Input: part model. Units: mm. Frame: model coordinates. A direction names the side the tool comes from. Give positions to 0.01 mm unless a question says otherwise; leave off trailing zeros. Loops run counter-clockwise (first coordinate to the right, second up) from the corner with the lowest first, then second, coordinate; pieces in that order, holes last. Notation, with made-up numbers: (-25.5, -17.75) - (-16.5, -17.75) arc R25 cw to (-16.5, -3.75) - close; hole circle Ø1 at (28.25, 75). An arc over 180 degrees is marked (long way). Answer as a JSON object with one key per item and string values. Group by question number.
(1) Access query for faces 5 (the flat face through (182, 0, -21)), 6 (the flat face through (184, -40, -5)). Directions: +Z, -Z, +X, -X, +Y, -Y. A direction counts if a zero-diameter tool reaches every point of the face in a straight line with its end or side. Return the directions, or none.
(2) Material intervals for L1, parallel to Z at x = 94.5, y = -63.5; L2, parallel to Y at x = 232, z = -37.5; L3, parallel to Y at x = 209, z = -15, sorted ascending.
(3) Pin query (flat end, axial travel): P1, Ø2, axis at x = 95.5, y = -23.5, coming from the -Z side. Return the tip coordinate at first contact, or that it passes through.
(4) Section query D-D (y = -13.5). Return loops of the section in (x, z), plus the area to 3 significant figures.
(5) Section query B-B (x = 260.5). Return loops of the section in (y, z), plus the area to 3 significant figures.
(6) Section query A-A (z = -27.5). Return loops of the section in (x, y), plus the area to 3 significant figures.
(7) Section query C-C (z = -14.5). Return loops of the section in (x, y), plus the area to 3 significant figures.
(8) Mould query, pull axis Y, two halves, no side actions, for faces 1 (the cylindrical face through (183.28, -11.711, -7.124)), 2 (the flat face through (300, -40, -4)), 3 (the flat face through (189.72, -72.16, -25.61)), 4 (the flat face through (190, -80, -22)). Classes: +Y half, -Y half, draft (parallel to the pull), parting line (faces both ways), or undercut.
```python
from build123d import *

# Parameters (mm, degrees)
GB_T707_1988_8_XXXXXXXXXXXXXXX528V9_1_DEPTH = 300
CUT_EXTRUDE_2_REACH                         = 315.447
SKETCH_4_R                                  = 895


with BuildPart() as part:
    # Sketch11 → 热轧普通槽钢(gb t707-1988) 8-XXXXXXXXXXXXXXX528V9(1) (new body)
    with BuildSketch(Plane(origin=(0, 0, 0), x_dir=(0, 0, -1), z_dir=(-1, 0, 0))):
        with BuildLine():
            Line((43, 80), (0, 80))
            Line((0, 80), (0, 0))
            Line((0, 0), (43, 0))
            Line((43, 0), (43, 2.480049752))
            ThreePointArc((43, 2.480049752), (41.965810134, 5.164071035), (39.398014876, 6.460198512))
            Line((39.398014876, 6.460198512), (12.203970248, 9.179602975))
            ThreePointArc((12.203970248, 9.179602975), (7.068379732, 11.771857931), (5, 17.139900497))
            Line((5, 17.139900497), (5, 62.860099503))
            ThreePointArc((5, 62.860099503), (7.068379732, 68.228142069), (12.203970248, 70.820397025))
            Line((12.203970248, 70.820397025), (39.398014876, 73.539801488))
            ThreePointArc((39.398014876, 73.539801488), (41.965810134, 74.835928965), (43, 77.519950248))
            Line((43, 77.519950248), (43, 80))
        make_face()
    extrude(amount=-GB_T707_1988_8_XXXXXXXXXXXXXXX528V9_1_DEPTH)

    # 草图4 → 切除-拉伸2 (cut, up to next)
    with BuildSketch(Plane.XY, mode=Mode.PRIVATE) as cut_extrude_2_sk1:
        with Locations((-799.887205022, -220.600173536)):
            Circle(SKETCH_4_R)
    cut_extrude_2_tool1 = extrude(cut_extrude_2_sk1.sketch, amount=-CUT_EXTRUDE_2_REACH, mode=Mode.PRIVATE) & part.part
    add(cut_extrude_2_tool1.solids().sort_by_distance((-799.887205, -220.600174, 0))[0], mode=Mode.SUBTRACT)


solid = part.part
```
Recorded:
{
 "1": {"face 5": "+Z, -Z, +X, -X, +Y", "face 6": "-Z, +X, -X"},
 "2": {"L1": "z = -5.03 to 0", "L2": "y = -80 to -73.35, -6.65 to 0", "L3": "y = -80 to -71.1, -8.9 to 0"},
 "3": {"P1": "stops at z = -5"},
 "4": {"outline": "(70.82, -5.88) - (300, -5.88) - (300, 0) - (70.82, 0) - close", "area": "1,350 mm^2"},
 "5": {"outline": "(-80, -43) - (-77.52, -43) arc R4 ccw to (-73.54, -39.4) - (-70.82, -12.2) arc R8 cw to (-62.86, -5) - (-17.14, -5) arc R8 cw to (-9.18, -12.2) - (-6.46, -39.4) arc R4 ccw to (-2.48, -43) - (0, -43) - (0, 0) - (-80, 0) - close", "area": "1,020 mm^2"},
 "6": {"outline": "(67.5, 0) arc R895 cw to (69.41, -7.65) - (300, -7.65) - (300, 0) - close; (82.75, -72.35) arc R895 cw to (84, -80) - (300, -80) - (300, -72.35) - close", "area": "3,430 mm^2"},
 "7": {"outline": "(67.5, 0) arc R895 cw to (69.73, -8.95) - (300, -8.95) - (300, 0) - close; (82.53, -71.05) arc R895 cw to (84, -80) - (300, -80) - (300, -71.05) - close", "area": "4,010 mm^2"},
 "8": {"face 1": "undercut", "face 2": "draft", "face 3": "undercut", "face 4": "-Y half"}
}
